Source: three-view drawing plus pictorial views. Frame: mm from the lowest corner of the part. A direction names the side the tool comes from. Give positions to 0.01 mm unless a question says otherwise; leave off trailing zeros. Order: outer loops, then holes, each group sorted by start corner. A loop starts at its lowest first (then second) coordinate and runs counter-clockwise, first axis right, second up. Notation, with made-up numbers: (-12, 61.5) -> (23, 61.5) arc R35 cw to (23, 95.5) -> close; hole circle Ø3 at (-2.5, 35). An arc over 180 degrees is marked (long way). Write item = value, one per line.
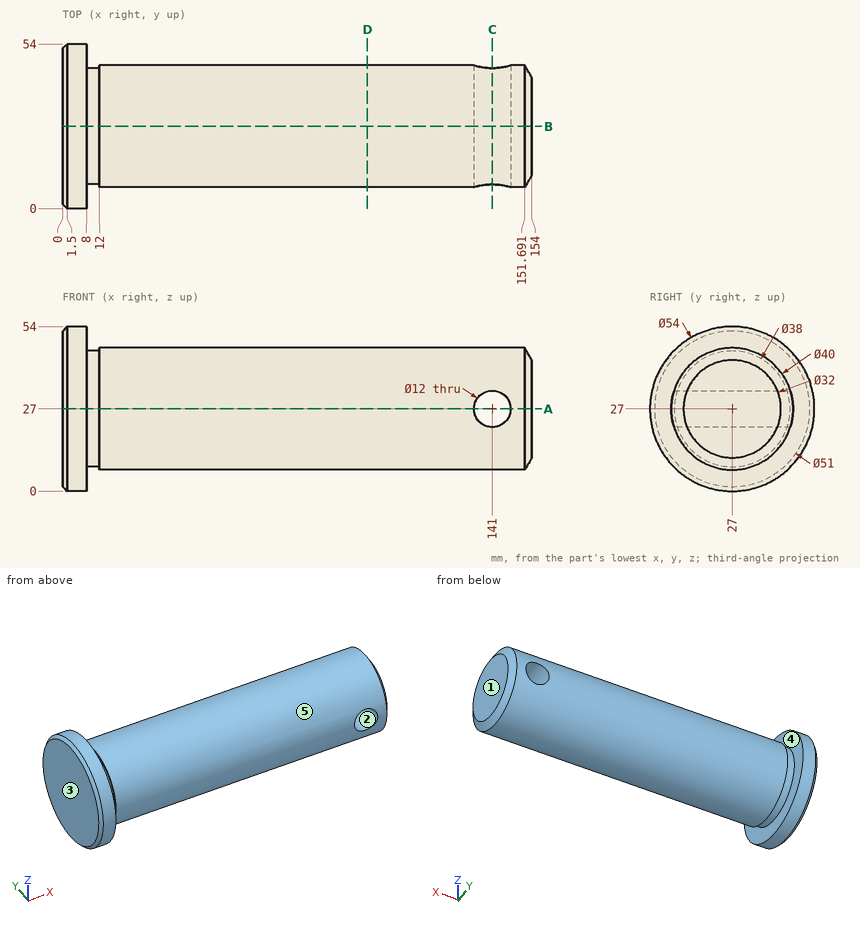
1) Section query B-B (y = 27). Output: boundary loops of the cut face in (x, z).
Check sheet entries:
outline = (0, 1.5) -> (1.5, 0) -> (8, 0) -> (8, 8) -> (12, 8) -> (12, 7) -> (151.69, 7) -> (154, 11) -> (154, 43) -> (151.69, 47) -> (12, 47) -> (12, 46) -> (8, 46) -> (8, 54) -> (1.5, 54) -> (0, 52.5) -> close; hole circle Ø12 at (141, 27)
2) Line query: line 1 (X direction, y = 16, z = 27); line 2 (Y direction, x = 43, z = 39); line 3 (X direction, y = 27, z = 5.5). Output: solid intervals per line, ascending. Write a range as from..to.
Check sheet entries:
line_1 = 0..135, 147..154
line_2 = 11..43
line_3 = 0..8
3) Reachability of the marked faces 4 and 5 from +Z, -Z, +X, -X, +Y, -Y: full face, straight path, thin tool, end or side. Return the list, or none.
Check sheet entries:
face_4 = none
face_5 = +X
4) Section query D-D (x = 100). Output: boundary loops of the cut face in (y, z), plus the area to 3 significant figures.
Check sheet entries:
outline = circle Ø40 at (27, 27)
area = 1,260 mm²
5) Section query A-A (z = 27). Output: boundary loops of the cut face in (x, y), plus the area to 3 significant figures.
Check sheet entries:
outline = (0, 1.5) -> (1.5, 0) -> (8, 0) -> (8, 8) -> (12, 8) -> (12, 7) -> (135, 7) -> (135, 47) -> (12, 47) -> (12, 46) -> (8, 46) -> (8, 54) -> (1.5, 54) -> (0, 52.5) -> close; (147, 7) -> (151.69, 7) -> (154, 11) -> (154, 43) -> (151.69, 47) -> (147, 47) -> close
area = 5,770 mm²
6) Section query C-C (x = 141). Output: boundary loops of the cut face in (y, z).
Check sheet entries:
outline = (7.92, 21) arc R20 ccw to (46.08, 21) -> close; (7.92, 33) -> (46.08, 33) arc R20 ccw to start
7) First-contact query: P1, Ø12, axis at x = 28, z = 20.5, coming from the +Y side; P2, Ø2, axis at x = 60, y = 14.5, coming from the -Z side; P3, Ø3, axis at x = 66, y = 18.5, coming from the -Z side (1 decimal). Flat tips, straight axial feed; report the tip coordinate or a pass-through.
Check sheet entries:
P1 = 46.99
P2 = 10.64
P3 = 8.3
8) Mould query, pull axis X, two halves, no side actions, for the marked faces 1, 2 and 3. Classes: +X half, -X half, draft (parallel to the pull), parting line (faces both ways), or undercut.
Check sheet entries:
face_1 = +X half
face_2 = undercut
face_3 = -X half
